```python
from build123d import *

# Parameters (mm, degrees)
SKETCH1_R           = 47
SKETCH1_R_2         = 10
SKETCH1_R_3         = 2.5
BOSS_EXTRUDE1_DEPTH = 5


with BuildPart() as part:
    # Sketch1 → Boss-Extrude1 (new body)
    with BuildSketch(Plane.XY):
        Circle(SKETCH1_R)
        Circle(SKETCH1_R_2, mode=Mode.SUBTRACT)
        with Locations((25, 0)):
            Circle(SKETCH1_R_3, mode=Mode.SUBTRACT)
        with Locations((-12.5, -21.650635095)):
            Circle(SKETCH1_R_3, mode=Mode.SUBTRACT)
        with Locations((-12.5, 21.650635095)):
            Circle(SKETCH1_R_3, mode=Mode.SUBTRACT)
    extrude(amount=BOSS_EXTRUDE1_DEPTH)


solid = part.part
```
Input: part model. Units: mm. Frame: model coordinates. Coordinates: 2 decimals unless noted, no trailing zeros. Loops run counter-clockwise (first coordinate to the right, second up) from the corner with the lowest first, then second, coordinate; pieces in that order, holes last. Notation, with made-up numbers: (-28.5, 29.5) -> (-24.5, 29.5) arc R15 cw to (-24.5, 39.5) -> close; hole circle Ø2 at (47, -16.75). An arc over 180 degrees is marked (long way). Use a Markdown table: item, result.
1) Cut plane D-D (z = 2.35). Return the cut outline in (x, y), then the cut area to 3 significant figures.
Results found:
| item | result |
|---|---|
| outline | circle Ø94 at (0, 0); hole circle Ø5 at (-12.5, -21.65); hole circle Ø5 at (-12.5, 21.65); hole circle Ø20 at (0, 0); hole circle Ø5 at (25, 0) |
| area | 6,570 mm2 |
2) Cut plane C-C (x = -12.5). Return the cut outline in (y, z), then the cut area to 3 significant figures.
Results found:
| item | result |
|---|---|
| outline | (-45.31, 0) -> (-24.15, 0) -> (-24.15, 5) -> (-45.31, 5) -> close; (-19.15, 0) -> (19.15, 0) -> (19.15, 5) -> (-19.15, 5) -> close; (24.15, 0) -> (45.31, 0) -> (45.31, 5) -> (24.15, 5) -> close |
| area | 403 mm2 |
3) Cut plane B-B (y = 0). Return the cut outline in (x, z), then the cut area to 3 significant figures.
Results found:
| item | result |
|---|---|
| outline | (-47, 0) -> (-10, 0) -> (-10, 5) -> (-47, 5) -> close; (10, 0) -> (22.5, 0) -> (22.5, 5) -> (10, 5) -> close; (27.5, 0) -> (47, 0) -> (47, 5) -> (27.5, 5) -> close |
| area | 345 mm2 |
4) Material intervals for line 1 along Y through (x, z) = (0, 2.6); line 2 along X through (y, z) = (-1, 2.25); line 3 along Y through (x, z) = (-12.5, 2.55), sorted ascending. Write a range as from..to.
Results found:
| item | result |
|---|---|
| line 1 | y = -47..-10, 10..47 |
| line 2 | x = -46.99..-9.95, 9.95..22.71, 27.29..46.99 |
| line 3 | y = -45.31..-24.15, -19.15..19.15, 24.15..45.31 |
5) Cut plane A-A (x = 0). Return the cut outline in (y, z), then the cut area to 3 significant figures.
Results found:
| item | result |
|---|---|
| outline | (-47, 0) -> (-10, 0) -> (-10, 5) -> (-47, 5) -> close; (10, 0) -> (47, 0) -> (47, 5) -> (10, 5) -> close |
| area | 370 mm2 |
6) Contact query for flat-ended pins moving along their axis: pin 1 (6 mm diameter, centred on x = -12.5, y = -21.65, fed in from -Z); pin 2 (1 mm diameter, centred on x = -13, z = 4.5, fed in from +Y); pin 3 (1 mm diameter, centred on y = 35.5, z = 0.5, fed in from +X); pin 4 (1 mm diameter, centred on y = -11.5, z = 3.5, fed in from +X). Output: stop coordinate, or through.
Results found:
| item | result |
|---|---|
| pin 1 | stops at z = 0 |
| pin 2 | stops at y = 45.31 |
| pin 3 | stops at x = 31.37 |
| pin 4 | stops at x = 45.69 |
7) Pull-direction query (Y, two-part tool) for faces 1 (the cylindrical face through (-2.17, -9.76, 2.46)), 2 (the flat face through (-1, 11, 0)), 3 (the cylindrical face through (44.83, 14.12, 2.46)); classes: released by +Y, released by -Y, zero draft, split by the parting line, or undercut.
Results found:
| item | result |
|---|---|
| face 1 | undercut |
| face 2 | zero draft |
| face 3 | split by the parting line |
